The model under review builds one solid part; all positions refer to its coordinate system, in mm. A direction names the side the tool comes from. Give positions to 0.01 mm unless a question says otherwise; leave off trailing zeros. Order: outer loops, then holes, each group sorted by start corner. A loop starts at its lowest first (then second) coordinate and runs counter-clockwise, first axis right, second up. Notation, with made-up numbers: (72, -37) -> (105, -37) arc R21 ccw to (105, -29) -> close; hole circle Ø3 at (82, -7). An arc over 180 degrees is marked (long way). Use one line per item in the form item = value.
```python
from build123d import *

# Parameters (mm, degrees)
SKETCH1_W           = 201
SKETCH1_H           = 17
BOSS_EXTRUDE1_DEPTH = 16


with BuildPart() as part:
    # Sketch1 → Boss-Extrude1 (new body)
    with BuildSketch(Plane(origin=(0, 0, 0), x_dir=(1, 0, 0), z_dir=(0, 1, 0))):
        Polygon((-125, 311.5), (-125, -311.5), (-100.5, -311.5), (-100.5, -294.5), (100.5, -294.5), (100.5, -311.5), (125, -311.5), (125, 311.5), (100.5, 311.5), (100.5, 294.5), (-100.5, 294.5), (-100.5, 311.5), align=None)
        with Locations((0, -157)):
            Rectangle(SKETCH1_W, SKETCH1_H, mode=Mode.SUBTRACT)
        with Locations((0, 157)):
            Rectangle(SKETCH1_W, SKETCH1_H, mode=Mode.SUBTRACT)
    extrude(amount=BOSS_EXTRUDE1_DEPTH)


solid = part.part
```
1. For pin 1 Ø8 at (x, y) = (22, 7) entering from -Z; pin 2 Ø1 at (x, y) = (87.5, 6.5) entering from +Z, all flat-tipped, find the tip position at first contact; note any pin that passes through.
Values:
pin_1 = -294.5
pin_2 = 294.5
2. Add section B-B on y = 11.5. Give the boundary of the cut face in (x, z).
Values:
outline = (-125, -311.5) -> (-100.5, -311.5) -> (-100.5, -294.5) -> (100.5, -294.5) -> (100.5, -311.5) -> (125, -311.5) -> (125, 311.5) -> (100.5, 311.5) -> (100.5, 294.5) -> (-100.5, 294.5) -> (-100.5, 311.5) -> (-125, 311.5) -> close; hole (-100.5, -165.5) -> (100.5, -165.5) -> (100.5, -148.5) -> (-100.5, -148.5) -> close; hole (-100.5, 148.5) -> (100.5, 148.5) -> (100.5, 165.5) -> (-100.5, 165.5) -> close
3. Add section A-A on x = -68.5. Give the boundary of the cut face in (y, z), then the cut area to 3 significant figures.
Values:
outline = (0, -294.5) -> (16, -294.5) -> (16, -165.5) -> (0, -165.5) -> close; (0, -148.5) -> (16, -148.5) -> (16, 148.5) -> (0, 148.5) -> close; (0, 165.5) -> (16, 165.5) -> (16, 294.5) -> (0, 294.5) -> close
area = 8,880 mm^2
4. The part is to be moulded in two halves that separate along X. For faces 6 (the face through (-125, 8, -4)), 7 (the face through (113, 8, -311.5)), 8 (the face through (-1, 8, 294.5)), say which applies: +X half, -X half, draft (parallel to the pull), parting line (faces both ways), or undercut.
Values:
face_6 = -X half
face_7 = draft
face_8 = undercut
5. For L1, parallel to Z at x = -66.5, y = 2.5; L2, parallel to X at y = 14.5, z = 152, list the stretches that pass through material, from the lowest coordinate up.
Values:
L1 = -294.5 to -165.5, -148.5 to 148.5, 165.5 to 294.5
L2 = -125 to -100.5, 100.5 to 125
6. Tool access review of faces 1 (the face through (100.5, 8, 303)), 2 (the face through (-1, 8, -165.5)), 3 (the face through (-100.5, 8, -303)), 4 (the face through (-2, 16, -4)), 5 (the face through (-2, 0, -4)): name each direction out of +Z, -Z, +X, -X, +Y, -Y from which nothing blocks a thin tool from reaching the whole face with its end or side.
Values:
face_1 = +Z, +Y, -Y
face_2 = +Y, -Y
face_3 = -Z, +Y, -Y
face_4 = +Z, -Z, +X, -X, +Y
face_5 = +Z, -Z, +X, -X, -Y
